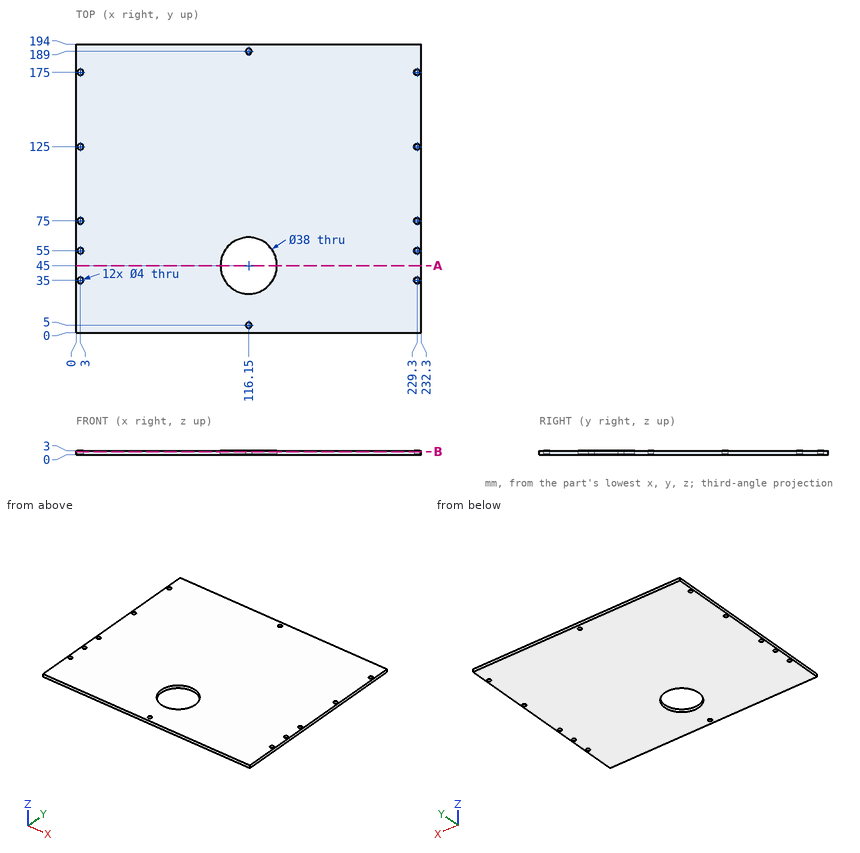
Check sheet for the drawn part. Datum: minimum x, y, z corner. Units: mm. Give positions to 0.01 mm unless a question says otherwise; leave off trailing zeros. Write each loop counter-clockwise with the first axis right and the second up, starting at its lowest first coordinate (ties: lowest second). Pieces come first, ordered by that corner, then holes.
(1) Cross-section at A-A (y = 45). Enter the section's corners in (x, z), plus the area to 3 significant figures.
(2) Material ranges on line 1 (Y direction, x = 229.3, z = 0.8); line 2 (Y direction, x = 116.15, z = 2.25); line 3 (X direction, y = 46, z = 1.7), recorded low to high.
(3) Cross-section at B-B (z = 2.3). State how many separate pieces and enclosed holes the cut face has, plus the area to 3 significant figures.
Worked out:
1. outline: (0, 0) - (97.15, 0) - (97.15, 3) - (0, 3) - close; (135.15, 0) - (232.3, 0) - (232.3, 3) - (135.15, 3) - close
1. area: 583 mm2
2. line 1: y = 0 to 33, 37 to 53, 57 to 73, 77 to 123, 127 to 173, 177 to 194
2. line 2: y = 0 to 3, 7 to 26, 64 to 187, 191 to 194
2. line 3: x = 0 to 97.18, 135.12 to 232.3
3. separate pieces: 1
3. enclosed holes: 13
3. area: 43,800 mm2
